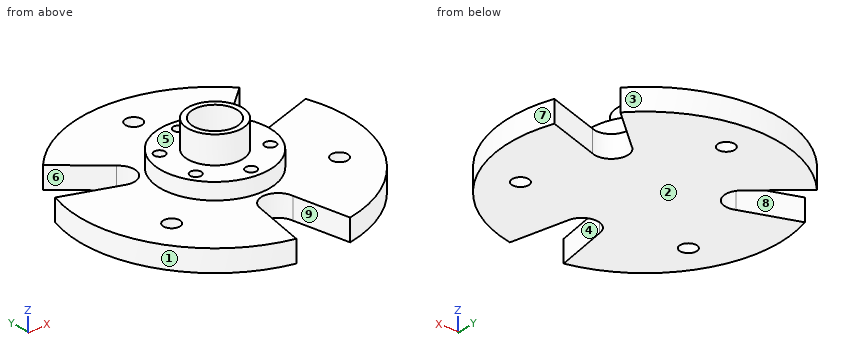
from build123d import *

# Parameters (mm, degrees)
FLANGE_PLATE_4MM_DEPTH   = 4
OUTER_HOLES_SKETCH_R     = 1.5
OUTER_HOLES_3X_DEPTH     = 35.855955648
HUB_SKETCH_R             = 10
RAISED_HUB_DEPTH         = 7
HUB_HOLES_SKETCH_R       = 1
HUB_HOLES_6X_DEPTH       = 3
CENTRE_SLEEVE_SKETCH_R   = 5
CENTRE_SLEEVE_SKETCH_R_2 = 4
CENTRE_SLEEVE_DEPTH      = 5


with BuildPart() as part:
    # Flange Plate Sketch → Flange Plate 4mm (new body)
    with BuildSketch(Plane.XY):
        with BuildLine():
            Line((-2.988714381, -13.67726531), (-5, -23.968079232))
            ThreePointArc((-5, -23.968079232), (-21.203811369, -12.242026202), (-23.256965495, 7.653912597))
            Line((-23.256965495, 7.653912597), (-13.339216403, 4.250330076))
            ThreePointArc((-13.339216403, 4.250330076), (-9.521006176, 5.496955479), (-10.350502022, 9.426935234))
            Line((-10.350502022, 9.426935234), (-18.256965495, 16.314166635))
            ThreePointArc((-18.256965495, 16.314166635), (0, 24.484052403), (18.256965495, 16.314166635))
            Line((18.256965495, 16.314166635), (10.350502022, 9.426935234))
            ThreePointArc((10.350502022, 9.426935234), (9.521006176, 5.496955479), (13.339216403, 4.250330076))
            Line((13.339216403, 4.250330076), (23.256965495, 7.653912597))
            ThreePointArc((23.256965495, 7.653912597), (21.203811369, -12.242026202), (5, -23.968079232))
            Line((5, -23.968079232), (2.988714381, -13.67726531))
            ThreePointArc((2.988714381, -13.67726531), (0, -10.993910957), (-2.988714381, -13.67726531))
        make_face()
    extrude(amount=FLANGE_PLATE_4MM_DEPTH)

    # Outer Holes Sketch → Outer Holes 3x (cut, through all)
    with BuildSketch(Plane.XY):
        with Locations((0, 18)):
            Circle(OUTER_HOLES_SKETCH_R)
        with Locations((15.588457268, -9)):
            Circle(OUTER_HOLES_SKETCH_R)
        with Locations((-15.588457268, -9)):
            Circle(OUTER_HOLES_SKETCH_R)
    extrude(amount=OUTER_HOLES_3X_DEPTH, mode=Mode.SUBTRACT)

    # Hub Sketch → Raised Hub (add)
    with BuildSketch(Plane.XY):
        Circle(HUB_SKETCH_R)
    extrude(amount=RAISED_HUB_DEPTH)

    # Hub Holes Sketch → Hub Holes 6x (cut)
    with BuildSketch(Plane.XY.offset(7)):
        with Locations((0, 8)):
            Circle(HUB_HOLES_SKETCH_R)
        with Locations((6.92870323, 4.000866025)):
            Circle(HUB_HOLES_SKETCH_R)
        with Locations((6.92970323, -3.999133975)):
            Circle(HUB_HOLES_SKETCH_R)
        with Locations((0.002, -8)):
            Circle(HUB_HOLES_SKETCH_R)
        with Locations((-6.92670323, -4.000866025)):
            Circle(HUB_HOLES_SKETCH_R)
        with Locations((-6.92770323, 3.999133975)):
            Circle(HUB_HOLES_SKETCH_R)
    extrude(amount=-HUB_HOLES_6X_DEPTH, mode=Mode.SUBTRACT)

    # Centre Sleeve Sketch → Centre Sleeve (add)
    with BuildSketch(Plane.XY.offset(7)):
        Circle(CENTRE_SLEEVE_SKETCH_R)
        Circle(CENTRE_SLEEVE_SKETCH_R_2, mode=Mode.SUBTRACT)
    extrude(amount=CENTRE_SLEEVE_DEPTH)


solid = part.part
The listing builds one solid part. Answer for the finished solid, in the listing's coordinates (mm). Face numbers are marked on the shaded views. A direction names the side the tool comes from. Give positions to 0.01 mm unless a question says otherwise; leave off trailing zeros. Write each loop counter-clockwise with the first axis right and the second up, starting at its lowest first coordinate (ties: lowest second). Pieces come first, ordered by that corner, then holes. Notation, with made-up numbers: (-8, 9.25) -> (17, 9.25) arc R19 ccw to (17, 45.25) -> close; hole circle Ø4 at (-30, 89). An arc over 180 degrees is marked (long way). Use a Markdown table: item, result.
(1) For the marked faces 5, 6, 7, 8 and 9, determine the directions among +Z, -Z, +X, -X, +Y, -Y from which every point of the face is accessible in a straight line to the end or side of a thin tool.
Return value:
| item | result |
|---|---|
| face 5 | +Z |
| face 6 | +Z, -Z, -X |
| face 7 | +Z, -Z, +X |
| face 8 | +Z, -Z |
| face 9 | +Z, -Z, -Y |
(2) Find the intervals of material crossed by probe 1 along Z at (x, y) = (10, -20.5); probe 2 along Y at (x, z) = (-14.5, 1.5); probe 3 along Z at (x, y) = (6, -5), in increasing order. Write a range as from..to.
Return value:
| item | result |
|---|---|
| probe 1 | 0..4 |
| probe 2 | -19.73..-10.03, -7.97..4.65, 13.04..19.73 |
| probe 3 | 0..7 |
(3) Determine the mould class of the marked faces 1, 2, 3 and 4 for opening direction X: released by +X, released by -X, zero draft, split by the parting line, or undercut.
Return value:
| item | result |
|---|---|
| face 1 | released by -X |
| face 2 | zero draft |
| face 3 | split by the parting line |
| face 4 | undercut |
(4) Section B-B, the plane x = 0 is taken. Determine the outline of the cut face in (y, z), then the cut area to 3 significant figures.
Return value:
| item | result |
|---|---|
| outline | (-10.99, 0) -> (16.5, 0) -> (16.5, 4) -> (10, 4) -> (10, 7) -> (9, 7) -> (9, 4) -> (7, 4) -> (7, 7) -> (5, 7) -> (5, 12) -> (4, 12) -> (4, 7) -> (-4, 7) -> (-4, 12) -> (-5, 12) -> (-5, 7) -> (-7, 7) -> (-7, 4) -> (-9, 4) -> (-9, 7) -> (-10, 7) -> (-10, 4) -> (-10.99, 4) -> close; (19.5, 0) -> (24.48, 0) -> (24.48, 4) -> (19.5, 4) -> close |
| area | 188 mm2 |
(5) Section D-D, the plane x = 16.5 is taken. Determine the outline of the cut face in (y, z), then the cut area to 3 significant figures.
Return value:
| item | result |
|---|---|
| outline | (-18.09, 0) -> (-10.19, 0) -> (-10.19, 4) -> (-18.09, 4) -> close; (-7.81, 0) -> (5.34, 0) -> (5.34, 4) -> (-7.81, 4) -> close; (14.78, 0) -> (18.09, 0) -> (18.09, 4) -> (14.78, 4) -> close |
| area | 97.4 mm2 |
(6) Section A-A, the plane z = 2.75 is taken. Determine the outline of the cut face in (x, y), then the cut area to 3 significant figures.
Return value:
| item | result |
|---|---|
| outline | (-23.26, 7.65) arc R24.48 ccw to (-5, -23.97) -> (-2.99, -13.68) arc R3.01 cw to (2.99, -13.68) -> (5, -23.97) arc R24.48 ccw to (23.26, 7.65) -> (13.34, 4.25) arc R3.01 cw to (10.35, 9.43) -> (18.26, 16.31) arc R24.48 ccw to (-18.26, 16.31) -> (-10.35, 9.43) arc R3.01 cw to (-13.34, 4.25) -> close; hole circle Ø3 at (-15.59, -9); hole circle Ø3 at (0, 18); hole circle Ø3 at (15.59, -9) |
| area | 1,570 mm2 |
(7) Flat-ended cylindrical pins translate along their axes: P1, Ø4, axis at x = -1.5, y = 0.5, coming from the +Z side; P2, Ø4, axis at x = 0, y = 18, coming from the +Z side; P3, Ø1, axis at x = -19, z = 1.5, coming from the +Y side. Find the tip coordinate at first contact, or state that the pin passes through.
Return value:
| item | result |
|---|---|
| P1 | z = 7 |
| P2 | z = 4 |
| P3 | y = 6.36 |
(8) Section C-C, the plane y = 0 is taken. Determine the outline of the cut face in (x, z), then the cut area to 3 significant figures.
Return value:
| item | result |
|---|---|
| outline | (-24.48, 0) -> (24.48, 0) -> (24.48, 4) -> (10, 4) -> (10, 7) -> (5, 7) -> (5, 12) -> (4, 12) -> (4, 7) -> (-4, 7) -> (-4, 12) -> (-5, 12) -> (-5, 7) -> (-10, 7) -> (-10, 4) -> (-24.48, 4) -> close |
| area | 266 mm2 |
